Answer from the drawing. Dimensions are ordinates in mm from the lowest x, y and z of the part. Coordinates: 2 decimals unless noted, no trailing zeros. Loops run counter-clockwise (first coordinate to the right, second up) from the corner with the lowest first, then second, coordinate; pieces in that order, holes last. Notation, with made-up numbers: (-27, -23) -> (1, -23) arc R21 cw to (1, -14) -> close; hole circle Ø4 at (72.5, 79). An arc over 180 degrees is marked (long way). Use a Markdown table: item, result.
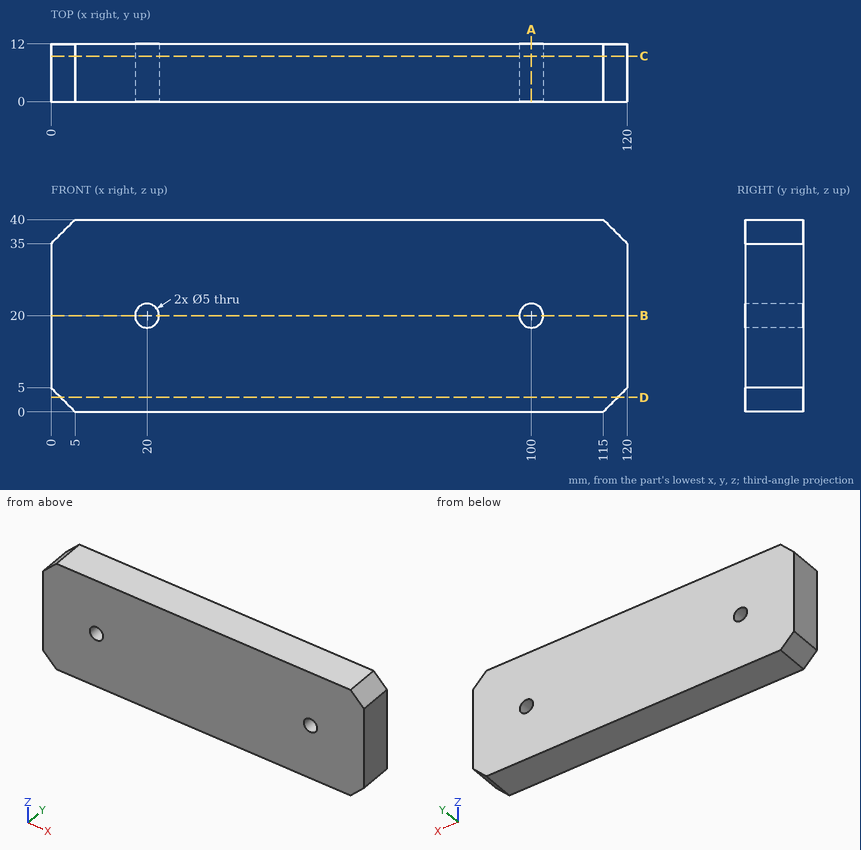
Q1. Section A-A on x = 100 is taken. Determine the outline of the cut face in (y, z).
Solved:
| item | result |
|---|---|
| outline | (0, 0) -> (12, 0) -> (12, 17.5) -> (0, 17.5) -> close; (0, 22.5) -> (12, 22.5) -> (12, 40) -> (0, 40) -> close |
Q2. Consider line 1 (Z direction, x = 100, y = 9.25); line 2 (X direction, y = 9.75, z = 18); line 3 (Z direction, x = 21.5, y = 4.5). Determine where each line is inside the solid, lowest interval first. Write a range as [from, to].
Solved:
| item | result |
|---|---|
| line 1 | [0, 17.5], [22.5, 40] |
| line 2 | [0, 18.5], [21.5, 98.5], [101.5, 120] |
| line 3 | [0, 18], [22, 40] |
Q3. Section C-C on y = 9.5 is taken. Determine the outline of the cut face in (x, z), and give its area (3 significant figures).
Solved:
| item | result |
|---|---|
| outline | (0, 5) -> (5, 0) -> (115, 0) -> (120, 5) -> (120, 35) -> (115, 40) -> (5, 40) -> (0, 35) -> close; hole circle Ø5 at (20, 20); hole circle Ø5 at (100, 20) |
| area | 4,710 mm² |
Q4. Section B-B on z = 20 is taken. Determine the outline of the cut face in (x, y).
Solved:
| item | result |
|---|---|
| outline | (0, 0) -> (17.5, 0) -> (17.5, 12) -> (0, 12) -> close; (22.5, 0) -> (97.5, 0) -> (97.5, 12) -> (22.5, 12) -> close; (102.5, 0) -> (120, 0) -> (120, 12) -> (102.5, 12) -> close |
Q5. Section D-D on z = 3 is taken. Determine the outline of the cut face in (x, y).
Solved:
| item | result |
|---|---|
| outline | (2, 0) -> (118, 0) -> (118, 12) -> (2, 12) -> close |
